from build123d import *

# Parameters (mm, degrees)
BOSS_EXTRUDE1_DEPTH   = 5
SKETCH2_R             = 2.5
CUT_EXTRUDE1_DEPTH    = 52.635743434
CHAMFER1_SIZE         = 0.5
CHAMFER2_SIZE         = 1
CHAMFER2_SIZE2        = 1.123603797
M5_TAPPED_HOLE1_D     = 4.2
M5_TAPPED_HOLE1_DEPTH = 26
M5_TAPPED_HOLE1_TIP   = 1.2618073


with BuildPart() as part:
    # Sketch1 → Boss-Extrude1 (new, symmetric)
    with BuildSketch(Plane.XY):
        Polygon((-40.5, -4), (-50.5, -2.948957647), (-50.5, 4), (50.5, 4), (50.5, -4), align=None)
    extrude(amount=BOSS_EXTRUDE1_DEPTH, both=True)

    # Sketch2 → Cut-Extrude1 (cut, through all)
    with BuildSketch(Plane.XY.offset(5)):
        with Locations((-45.5, 0)):
            Circle(SKETCH2_R)
        with Locations((24.5, 0)):
            Circle(SKETCH2_R)
    extrude(amount=-CUT_EXTRUDE1_DEPTH, mode=Mode.SUBTRACT)

    # Chamfer1
    chamfer1_edges = [part.edges().sort_by_distance(p)[0] for p in [
        (5, -4, 5),
        (5, -4, -5),
        (0, 4, -5),
        (0, 4, 5),
        (50.5, -4, 0),
        (-50.5, 4, 0),
        (50.5, 4, 0),
    ]]
    chamfer(chamfer1_edges, length=CHAMFER1_SIZE)

    # Chamfer2
    chamfer2_edges = [part.edges().sort_by_distance(p)[0] for p in [
        (-50.5, -2.948957647, 0),
    ]]
    chamfer2_side = [part.faces().sort_by_distance(p)[0] for p in [
        (-50.5, 0.275521176, 0),
    ]]
    chamfer(chamfer2_edges, length=CHAMFER2_SIZE, length2=CHAMFER2_SIZE2, reference=chamfer2_side[0])

    # M5 Tapped Hole1
    with Locations(Plane(origin=(50.5, 0, 0), x_dir=(0, 0, -1), z_dir=(1, 0, 0))):
        with Locations((0, 0)):
            Hole(M5_TAPPED_HOLE1_D / 2, depth=M5_TAPPED_HOLE1_DEPTH)
            with Locations((0, 0, -(M5_TAPPED_HOLE1_DEPTH + M5_TAPPED_HOLE1_TIP / 2))):  # 118° drill point
                Cone(0, M5_TAPPED_HOLE1_D / 2, M5_TAPPED_HOLE1_TIP, mode=Mode.SUBTRACT)


solid = part.part
The model under review builds one solid part; all positions refer to its coordinate system, in mm. Give positions to 0.01 mm unless a question says otherwise; leave off trailing zeros. Loops run counter-clockwise (first coordinate to the right, second up) from the corner with the lowest first, then second, coordinate; pieces in that order, holes last. Notation, with made-up numbers: (67, 32.25) -> (90, 32.25) arc R20 ccw to (90, 63.25) -> close; hole circle Ø8 at (78.25, 21). An arc over 180 degrees is marked (long way). Write each question's results on one line, items separated by ' | '.
1) For line 1 along X through (y, z) = (-0.25, 2); line 2 along Z through (x, y) = (38.25, 0); line 3 along X through (y, z) = (-2, 4.5), list the stretches that pass through material, from the lowest coordinate up. Write a range as from..to.
Conclusion:
line 1: x = -50.5..-47.99, -43.01..22.01 | line 2: z = -5..-2.1, 2.1..5 | line 3: x = -50.45..-47, -44..23, 26..50.5
2) Draft analysis for pull direction Z (two halves, no side actions). For faces 1 (the face through (50.5, 0, 2.3)), 2 (the face through (38.006, 0.631, 2.003)), 3 (the face through (1, 0, -5)), 4 (the face through (1, 0, 5)), state which applies: pulls with the +Z half, pulls with the -Z half, needs draft (parallel to the pull), parting line crosses it, or undercut.
Conclusion:
face 1: needs draft | face 2: undercut | face 3: pulls with the -Z half | face 4: pulls with the +Z half
3) Take a section at B-B, the plane z = 3. Give the boundary of the cut face in (x, y).
Conclusion:
outline: (-50.5, -1.95) -> (-49.38, -3.07) -> (-40.5, -4) -> (50, -4) -> (50.5, -3.5) -> (50.5, 3.5) -> (50, 4) -> (-50, 4) -> (-50.5, 3.5) -> close; hole circle Ø5 at (-45.5, 0); hole circle Ø5 at (24.5, 0)
4) Take a section at A-A, the plane x = 24.5. Give the boundary of the cut face in (y, z).
Conclusion:
outline: (-4, -4.5) -> (-3.5, -5) -> (-2.5, -5) -> (-2.5, 5) -> (-3.5, 5) -> (-4, 4.5) -> close; (2.5, -5) -> (3.5, -5) -> (4, -4.5) -> (4, 4.5) -> (3.5, 5) -> (2.5, 5) -> close
5) Take a section at C-C, the plane y = 0. Give the boundary of the cut face in (x, z).
Conclusion:
outline: (-50.5, -5) -> (-48, -5) -> (-48, 5) -> (-50.5, 5) -> close; (-43, -5) -> (22, -5) -> (22, 5) -> (-43, 5) -> close; (27, -5) -> (50.5, -5) -> (50.5, -2.1) -> (27, -2.1) -> close; (27, 2.1) -> (50.5, 2.1) -> (50.5, 5) -> (27, 5) -> close
6) Insertion check: pin 1 Ø2.5 at (y, z) = (0, 0) entering from +X; pin 2 Ø4 at (x, y) = (-45.5, 0) entering from -Z; pin 3 Ø1 at (x, y) = (25, 2) entering from -Z. Each pin has a flat end and moves straight along its axis. Give the tip position at first contact, or say it passes through.
Conclusion:
pin 1: stops at x = 22.33 | pin 2: passes through | pin 3: stops at z = -5
7) Take a section at D-D, the plane z = -1.25. Give the boundary of the cut face in (x, y).
Conclusion:
outline: (-50.5, -1.95) -> (-49.38, -3.07) -> (-40.5, -4) -> (50, -4) -> (50.5, -3.5) -> (50.5, -1.69) -> (26.34, -1.69) arc R2.5 cw (long way) to (26.34, 1.69) -> (50.5, 1.69) -> (50.5, 3.5) -> (50, 4) -> (-50, 4) -> (-50.5, 3.5) -> close; hole circle Ø5 at (-45.5, 0)
